from build123d import *

# Parameters (mm, degrees)
EXTRUDE_1_DEPTH     = 31.5
SKETCH_2_W          = 29
SKETCH_2_H          = 63
CUT_EXTRUDE_1_DEPTH = 1.5
CUT_EXTRUDE_2_DEPTH = 0.3
HOLE_WIZARD_M5_1_D  = 4.2


with BuildPart() as part:
    # 草图1 → 凸台-拉伸1 (new, symmetric)
    with BuildSketch(Plane.XY):
        Polygon((0, 0), (32, 0), (32, -30), (22, -30), (22, -20), (0, -20), align=None)
    extrude(amount=EXTRUDE_1_DEPTH, both=True)

    # 草图2 → 切除-拉伸1 (cut)
    with BuildSketch(Plane(origin=(0, 0, 0), x_dir=(1, 0, 0), z_dir=(0, 1, 0))):
        with Locations((17.5, 0)):
            Rectangle(SKETCH_2_W, SKETCH_2_H)
    extrude(amount=-CUT_EXTRUDE_1_DEPTH, mode=Mode.SUBTRACT)

    # 草图3 → 切除-拉伸2 (cut)
    with BuildSketch(Plane(origin=(32, 0, 0), x_dir=(0, 0, -1), z_dir=(1, 0, 0))):
        Polygon((-16.814964409, -1.5), (-6.814964409, -30), (16.5, -30), (6.5, -1.5), align=None)
    extrude(amount=-CUT_EXTRUDE_2_DEPTH, mode=Mode.SUBTRACT)

    # M5 螺纹孔1 (through all)
    with Locations(Plane(origin=(31.7, -23, -2.386377444), x_dir=(0, 0, 1), z_dir=(1, 0, 0))):
        with Locations((0, 0)):
            Hole(HOLE_WIZARD_M5_1_D / 2)


solid = part.part
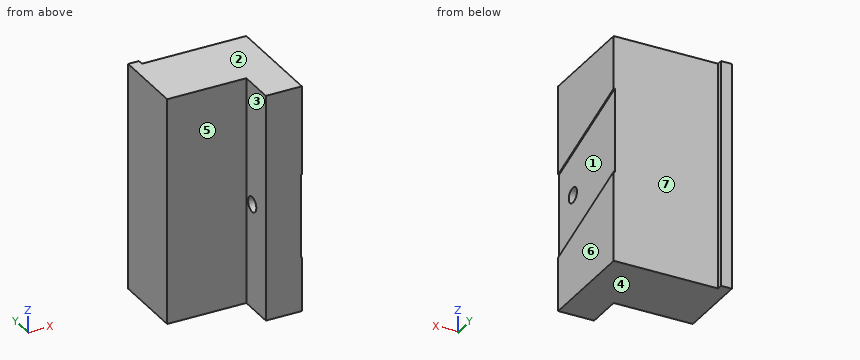
Part model, mm, in its own coordinate system. Face numbers are marked on the shaded views. A direction names the side the tool comes from. Give positions to 0.01 mm unless a question says otherwise; leave off trailing zeros. Order: outer loops, then holes, each group sorted by start corner. A loop starts at its lowest first (then second) coordinate and runs counter-clockwise, first axis right, second up. Notation, with made-up numbers: (65.25, -3) - (100.25, -3) arc R28 ccw to (100.25, 33) - close; hole circle Ø5 at (82, 30). An arc over 180 degrees is marked (long way). One line per question, with ' | ' between items.
1. Drop flat-ended pins along their axis: P1, Ø3, axis at y = -26, z = 3.5, coming from the -X side; P2, Ø4, axis at x = 14.5, z = -8.5, coming from the -Y side; P3, Ø1.5, axis at x = 5, z = 10.5, coming from the +Y side. Give the stop position or say it passes through.
Filled in:
P1: x = 22 | P2: y = -20 | P3: y = -1.5
2. Band-saw the part on B-B on x = 24.5. List the corners of the cut face in (y, z).
Filled in:
outline: (-30, -31.5) - (-1.5, -31.5) - (-1.5, 31.5) - (-30, 31.5) - close; hole circle Ø4.2 at (-23, -2.39)
3. Band-saw the part on D-D on z = 1. List the corners of the cut face in (x, y), then the cut area to 3 significant figures.
Filled in:
outline: (0, -20) - (22, -20) - (22, -30) - (31.7, -30) - (31.7, -1.5) - (3, -1.5) - (3, 0) - (0, 0) - close | area: 688 mm²
4. Band-saw the part on A-A on z = 25. List the corners of the cut face in (x, y), then the cut area to 4 significant figures.
Filled in:
outline: (0, -20) - (22, -20) - (22, -30) - (32, -30) - (32, -1.5) - (3, -1.5) - (3, 0) - (0, 0) - close | area: 696.5 mm²
5. Drill centre lines: probe 1 along Z at (x, y) = (29.25, -23); probe 2 along Y at (x, z) = (13.5, -2); probe 3 along X at (y, z) = (-21, -27). Where is each one in solid material? Low to high.
Filled in:
probe 1: -31.5 to -4.49, -0.29 to 31.5 | probe 2: -20 to -1.5 | probe 3: 22 to 32
6. Which spindle directions (+Z, -Z, +X, -X, +Y, -Y) get a long thin tool onto all of the face, cutting with end or side? Do the marked faces 5, 6 and 7. Say none if no direction does.
Filled in:
face 5: +Z, -Z, -X, -Y | face 6: +Z, -Z, +X, +Y, -Y | face 7: +Z, -Z, +X, +Y
7. Band-saw the part on C-C on y = -23. List the corners of the cut face in (x, z).
Filled in:
outline: (22, -31.5) - (32, -31.5) - (32, -14.04) - (31.7, -14.04) - (31.7, -4.49) - (22, -4.49) - close; (22, -0.29) - (31.7, -0.29) - (31.7, 9.27) - (32, 9.27) - (32, 31.5) - (22, 31.5) - close
8. Pull direction Z, two halves, no side cores. Call the marked faces 1, 2, 3 and 4: +Z half, -Z half, draft (parallel to the pull), parting line (faces both ways), or undercut.
Filled in:
face 1: undercut | face 2: +Z half | face 3: draft | face 4: -Z half
